Input: part model. Units: mm. Frame: model coordinates. Face numbers are marked on the shaded views. A direction names the side the tool comes from. Round coordinates to 2 decimals unless told otherwise and drop trailing zeros. Loops run counter-clockwise (first coordinate to the right, second up) from the corner with the lowest first, then second, coordinate; pieces in that order, holes last. Notation, with made-up numbers: (80, -19.5) -> (105, -19.5) arc R24 ccw to (105, -0.5) -> close; hole circle Ø6 at (48.5, -11.75). An arc over 180 degrees is marked (long way). Answer as a JSON object with one key per item and string values.
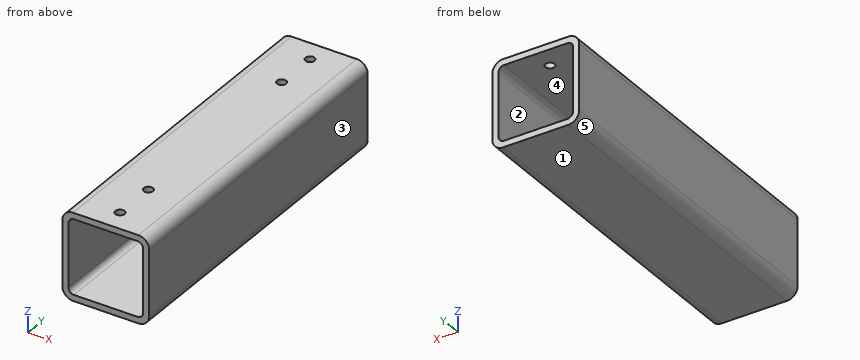
```python
from build123d import *

# Parameters (mm, degrees)
SKETCH1_W                      = 307.64
SKETCH1_H                      = 80
BOSS_EXTRUDE1_DEPTH            = 80
SKETCH2_W                      = 68.6
SKETCH2_H                      = 68.6
CUT_EXTRUDE1_DEPTH             = 314.476266406
F_8_5_8_5_DIAMETER_HOLE2_D     = 8.5
F_8_5_8_5_DIAMETER_HOLE2_DEPTH = 5.7
FILLET1_R                      = 5
FILLET2_R                      = 10
F_8_5_8_5_DIAMETER_HOLE3_D     = 8.5
F_8_5_8_5_DIAMETER_HOLE3_DEPTH = 10
F_8_5_8_5_DIAMETER_HOLE3_TIP   = 2.553657631
F_8_5_8_5_DIAMETER_HOLE5_D     = 8.5
F_8_5_8_5_DIAMETER_HOLE5_DEPTH = 10
F_8_5_8_5_DIAMETER_HOLE5_TIP   = 2.553657631


with BuildPart() as part:
    # Sketch1 → Boss-Extrude1 (new body)
    with BuildSketch(Plane(origin=(-35, 0, 0), x_dir=(0, -1, 0), z_dir=(-1, 0, 0))):
        with Locations((95.322857143, 0)):
            Rectangle(SKETCH1_W, SKETCH1_H)
    extrude(amount=-BOSS_EXTRUDE1_DEPTH)

    # Sketch2 → Cut-Extrude1 (cut, through all)
    with BuildSketch(Plane.XZ.offset(249.142857143)):
        with Locations((5, 0)):
            Rectangle(SKETCH2_W, SKETCH2_H)
    extrude(amount=-CUT_EXTRUDE1_DEPTH, mode=Mode.SUBTRACT)

    # Ø8.5 (8.5) Diameter Hole2
    with Locations(Plane.XY.offset(40)):
        with Locations((5, -189.142857143), (5, -229.142857143)):
            Hole(F_8_5_8_5_DIAMETER_HOLE2_D / 2, depth=F_8_5_8_5_DIAMETER_HOLE2_DEPTH)

    # Fillet1
    fillet1_edges = [part.edges().sort_by_distance(p)[0] for p in [
        (-29.3, -95.322857143, -34.3),
        (-29.3, -95.322857143, 34.3),
        (39.3, -95.322857143, 34.3),
        (39.3, -95.322857143, -34.3),
    ]]
    fillet(fillet1_edges, radius=FILLET1_R)

    # Fillet2
    fillet2_edges = [part.edges().sort_by_distance(p)[0] for p in [
        (45, -95.322857143, 40),
        (45, -95.322857143, -40),
        (-35, -95.322857143, 40),
        (-35, -95.322857143, -40),
    ]]
    fillet(fillet2_edges, radius=FILLET2_R)

    # Ø8.5 (8.5) Diameter Hole3
    with Locations(Plane.XY.offset(40)):
        with Locations((5, 38.497142857)):
            Hole(F_8_5_8_5_DIAMETER_HOLE3_D / 2, depth=F_8_5_8_5_DIAMETER_HOLE3_DEPTH)
            with Locations((0, 0, -(F_8_5_8_5_DIAMETER_HOLE3_DEPTH + F_8_5_8_5_DIAMETER_HOLE3_TIP / 2))):  # 118° drill point
                Cone(0, F_8_5_8_5_DIAMETER_HOLE3_D / 2, F_8_5_8_5_DIAMETER_HOLE3_TIP, mode=Mode.SUBTRACT)

    # Ø8.5 (8.5) Diameter Hole5
    with Locations(Plane.XY.offset(40)):
        with Locations((5, -1.502857143)):
            Hole(F_8_5_8_5_DIAMETER_HOLE5_D / 2, depth=F_8_5_8_5_DIAMETER_HOLE5_DEPTH)
            with Locations((0, 0, -(F_8_5_8_5_DIAMETER_HOLE5_DEPTH + F_8_5_8_5_DIAMETER_HOLE5_TIP / 2))):  # 118° drill point
                Cone(0, F_8_5_8_5_DIAMETER_HOLE5_D / 2, F_8_5_8_5_DIAMETER_HOLE5_TIP, mode=Mode.SUBTRACT)


solid = part.part
```
1) Draft query along Z for the marked faces 1, 2 and 3. Return one class per face: +Z half, -Z half, draft (parallel to the pull), parting line (faces both ways), or undercut.
Output:
{"face 1": "-Z half", "face 2": "undercut", "face 3": "draft"}
2) Ray query, probe 1 along Y at (x, z) = (5, 35); probe 2 along Z at (x, y) = (4.5, -142); probe 3 along X at (y, z) = (26, -6.5). Return the intervals inside material, ascending.
Output:
{"probe 1": "y = -249.14 to -233.39, -224.89 to -193.39, -184.89 to -5.75, 2.75 to 34.25, 42.75 to 58.5", "probe 2": "z = -40 to -34.3, 34.3 to 40", "probe 3": "x = -35 to -29.3, 39.3 to 45"}
3) Section B-B, the plane z = 20.5. Output: boundary loops of the cut face in (x, y).
Output:
{"outline": "(-35, -249.14) -> (-29.3, -249.14) -> (-29.3, 58.5) -> (-35, 58.5) -> close; (39.3, -249.14) -> (45, -249.14) -> (45, 58.5) -> (39.3, 58.5) -> close"}
4) Section D-D, the plane x = 28. Output: boundary loops of the cut face in (y, z).
Output:
{"outline": "(-249.14, -40) -> (58.5, -40) -> (58.5, -34.3) -> (-249.14, -34.3) -> close; (-249.14, 34.3) -> (58.5, 34.3) -> (58.5, 40) -> (-249.14, 40) -> close"}
5) Reachability of the marked faces 4 and 5 from +Z, -Z, +X, -X, +Y, -Y: full face, straight path, thin tool, end or side. Return the list, or none.
Output:
{"face 4": "+Y, -Y", "face 5": "-Z, -X, +Y, -Y"}
6) Section C-C, the plane y = -133. Output: boundary loops of the cut face in (x, z).
Output:
{"outline": "(-35, -30) arc R10 ccw to (-25, -40) -> (35, -40) arc R10 ccw to (45, -30) -> (45, 30) arc R10 ccw to (35, 40) -> (-25, 40) arc R10 ccw to (-35, 30) -> close; hole (-29.3, -29.3) arc R5 ccw to (-24.3, -34.3) -> (34.3, -34.3) arc R5 ccw to (39.3, -29.3) -> (39.3, 29.3) arc R5 ccw to (34.3, 34.3) -> (-24.3, 34.3) arc R5 ccw to (-29.3, 29.3) -> close"}
7) Section A-A, the plane x = 5. Output: boundary loops of the cut face in (y, z).
Output:
{"outline": "(-249.14, -40) -> (58.5, -40) -> (58.5, -34.3) -> (-249.14, -34.3) -> close; (-249.14, 34.3) -> (-233.39, 34.3) -> (-233.39, 40) -> (-249.14, 40) -> close; (-224.89, 34.3) -> (-193.39, 34.3) -> (-193.39, 40) -> (-224.89, 40) -> close; (-184.89, 34.3) -> (-5.75, 34.3) -> (-5.75, 40) -> (-184.89, 40) -> close; (2.75, 34.3) -> (34.25, 34.3) -> (34.25, 40) -> (2.75, 40) -> close; (42.75, 34.3) -> (58.5, 34.3) -> (58.5, 40) -> (42.75, 40) -> close"}
8) Contact query for a flat-ended pin moving along its axis: P1, Ø5, axis at x = 5, y = -189.14, coming from the +Z side. Output: stop coordinate, or through.
Output:
{"P1": "stops at z = -34.3"}
